Build history of the part. All positions in model axes, mm. Give positions to 0.01 mm unless a question says otherwise; leave off trailing zeros. Loops run counter-clockwise (first coordinate to the right, second up) from the corner with the lowest first, then second, coordinate; pieces in that order, holes last. Notation, with made-up numbers: M 23,35 L 68,35 A25 cw 68,66 Z; hole C 10,10 d11. An arc over 180 degrees is marked long. Put each result on its own line as item: value.
```python
from build123d import *

# Parameters (mm, degrees)
SKETCH1_W           = 36
SKETCH1_H           = 580
BOSS_EXTRUDE1_DEPTH = 16
CUT_EXTRUDE1_DEPTH  = 581.424844403
CUT_EXTRUDE2_DEPTH  = 291.848757948


with BuildPart() as part:
    # Sketch1 → Boss-Extrude1 (new body)
    with BuildSketch(Plane(origin=(0, 13, 0), x_dir=(1, 0, 0), z_dir=(0, 1, 0))):
        Rectangle(SKETCH1_W, SKETCH1_H)
    extrude(amount=-BOSS_EXTRUDE1_DEPTH)

    # Sketch2 → Cut-Extrude1 (cut, through all)
    with BuildSketch(Plane(origin=(0, 0, -290), x_dir=(-1, 0, 0), z_dir=(0, 0, -1))):
        Polygon((12, -3), (12, 0), (15, 0), (15, 10), (-15, 10), (-15, 0), (-12, 0), (-12, -3), align=None)
    extrude(amount=-CUT_EXTRUDE1_DEPTH, mode=Mode.SUBTRACT)

    # Sketch3 → Cut-Extrude2 (cut, through all)
    with BuildSketch(Plane.XZ.offset(-10)):
        with BuildLine():
            Line((10, -250), (10, 250))
            ThreePointArc((10, 250), (0, 260), (-10, 250))
            Line((-10, 250), (-10, -250))
            ThreePointArc((-10, -250), (0, -260), (10, -250))
        make_face()
    extrude(amount=-CUT_EXTRUDE2_DEPTH, mode=Mode.SUBTRACT)


solid = part.part
```
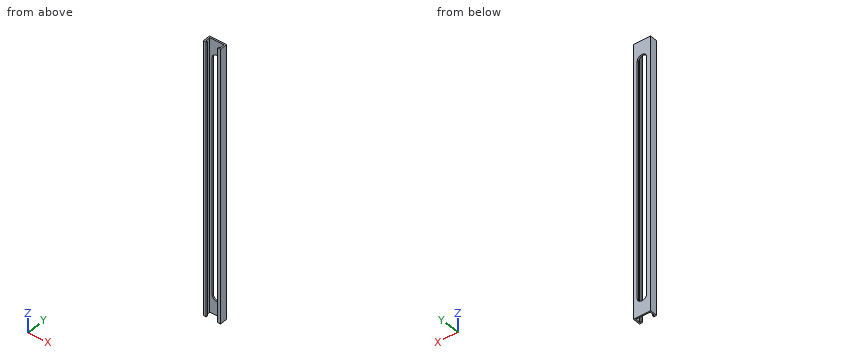
Q1. Slice it at B-B (z = -240). List the corners of the cut face in (x, y).
Here are the results:
outline: M -18,-3 L -12,-3 L -12,0 L -15,0 L -15,10 L -10,10 L -10,13 L -18,13 Z; M 10,10 L 15,10 L 15,0 L 12,0 L 12,-3 L 18,-3 L 18,13 L 10,13 Z
Q2. Probe line 1 (Y direction, x = -13, z = -165); line 2 (X direction, y = 8, z = 257.5); line 3 (X direction, y = 10.25, z = -177). List the from-to ranges inside material, lowest first. Write a range as from..to.
Here are the results:
line 1: -3..0, 10..13
line 2: -18..-15, 15..18
line 3: -18..-10, 10..18
Q3. Slice it at A-A (x = 0). List the corners of the cut face in (y, z).
Here are the results:
outline: M 10,-290 L 13,-290 L 13,-260 L 10,-260 Z; M 10,260 L 13,260 L 13,290 L 10,290 Z
Q4. Slice it at C-C (y = 4.5). List the corners of the cut face in (x, z).
Here are the results:
outline: M -18,-290 L -15,-290 L -15,290 L -18,290 Z; M 15,-290 L 18,-290 L 18,290 L 15,290 Z
